from build123d import *

# Parameters (mm, degrees)
SKETCH1_W             = 50
SKETCH1_H             = 20
BOSS_EXTRUDE1_DEPTH   = 100
SKETCH2_R             = 3
BOSS_EXTRUDE2_DEPTH   = 5
M6_TAPPED_HOLE1_D     = 5
M6_TAPPED_HOLE1_DEPTH = 15
M6_TAPPED_HOLE1_TIP   = 1.502151548
SKETCH5_W             = 20
SKETCH5_H             = 30
BOSS_EXTRUDE3_DEPTH   = 120
M3_TAPPED_HOLE1_D     = 2.5
M3_TAPPED_HOLE1_DEPTH = 7.5
M3_TAPPED_HOLE1_TIP   = 0.751075774
SKETCH8_W             = 147.482871738
SKETCH8_H             = 30
CUT_EXTRUDE1_DEPTH    = 163.249807396
SKETCH9_R             = 3
BOSS_EXTRUDE4_DEPTH   = 5
M6_TAPPED_HOLE2_D     = 5
M6_TAPPED_HOLE2_DEPTH = 15
M6_TAPPED_HOLE2_TIP   = 1.502151548


with BuildPart() as part:
    # Sketch1 → Boss-Extrude1 (new body)
    with BuildSketch(Plane(origin=(0, 0, 0), x_dir=(1, 0, 0), z_dir=(0, 1, 0))):
        Rectangle(SKETCH1_W, SKETCH1_H)
    extrude(amount=BOSS_EXTRUDE1_DEPTH)

    # Sketch2 → Boss-Extrude2 (add)
    with BuildSketch(Plane.XZ):
        with Locations(Location((0, 5, 0), (0, 0, 270))):
            Circle(SKETCH2_R)
    extrude(amount=BOSS_EXTRUDE2_DEPTH)

    # M6 Tapped Hole1
    with Locations(Plane(origin=(0, 0, 0), x_dir=(-1, 0, 0), z_dir=(0, -1, 0))):
        with Locations((0, 5)):
            Hole(M6_TAPPED_HOLE1_D / 2, depth=M6_TAPPED_HOLE1_DEPTH)
            with Locations((0, 0, -(M6_TAPPED_HOLE1_DEPTH + M6_TAPPED_HOLE1_TIP / 2))):  # 118° drill point
                Cone(0, M6_TAPPED_HOLE1_D / 2, M6_TAPPED_HOLE1_TIP, mode=Mode.SUBTRACT)

    # Sketch5 → Boss-Extrude3 (add)
    with BuildSketch(Plane(origin=(25, 0, 0), x_dir=(0, 0, -1), z_dir=(1, 0, 0))):
        with Locations((0, 115)):
            Rectangle(SKETCH5_W, SKETCH5_H)
    extrude(amount=-BOSS_EXTRUDE3_DEPTH)

    # M3 Tapped Hole1
    with Locations(Plane.XY.offset(10)):
        with Locations((-63.4, 108), (-59.4, 112), (-67.4, 105)):
            Hole(M3_TAPPED_HOLE1_D / 2, depth=M3_TAPPED_HOLE1_DEPTH)
            with Locations((0, 0, -(M3_TAPPED_HOLE1_DEPTH + M3_TAPPED_HOLE1_TIP / 2))):  # 118° drill point
                Cone(0, M3_TAPPED_HOLE1_D / 2, M3_TAPPED_HOLE1_TIP, mode=Mode.SUBTRACT)

    # Sketch8 → Cut-Extrude1 (cut, through all)
    with BuildSketch(Plane.XY.offset(10)):
        with Locations((-48.741435869, 115)):
            Rectangle(SKETCH8_W, SKETCH8_H)
    extrude(amount=-CUT_EXTRUDE1_DEPTH, mode=Mode.SUBTRACT)

    # Sketch9 → Boss-Extrude4 (add)
    with BuildSketch(Plane(origin=(0, 100, 0), x_dir=(1, 0, 0), z_dir=(0, 1, 0))):
        with Locations((-10, 0)):
            Circle(SKETCH9_R)
    extrude(amount=BOSS_EXTRUDE4_DEPTH)

    # M6 Tapped Hole2
    with Locations(Plane(origin=(0, 100, 0), x_dir=(1, 0, 0), z_dir=(0, 1, 0))):
        with Locations((0, 0)):
            Hole(M6_TAPPED_HOLE2_D / 2, depth=M6_TAPPED_HOLE2_DEPTH)
            with Locations((0, 0, -(M6_TAPPED_HOLE2_DEPTH + M6_TAPPED_HOLE2_TIP / 2))):  # 118° drill point
                Cone(0, M6_TAPPED_HOLE2_D / 2, M6_TAPPED_HOLE2_TIP, mode=Mode.SUBTRACT)


solid = part.part
Geometry check sheet. Reference: the model listing, model coordinates, mm. A direction names the side the tool comes from. Give positions to 0.01 mm unless a question says otherwise; leave off trailing zeros. Write each loop counter-clockwise with the first axis right and the second up, starting at its lowest first coordinate (ties: lowest second). Pieces come first, ordered by that corner, then holes.
1) Release check for a two-part mould opening along X. For faces 3 (the face through (0.54, 92.4, 2.44)), 4 (the face through (-12.4, 102.5, 1.8)), 5 (the face through (0, 0, 0)) record: released by +X, released by -X, zero draft, split by the parting line, or undercut.
Values follow:
face 3: undercut
face 4: split by the parting line
face 5: zero draft
2) Go/stop test with flat-tipped pins: pin 1 Ø5 at (x, z) = (15, 0.5) entering from +Y; pin 2 Ø2 at (x, z) = (12, 7.5) entering from -Y. Record where each tip stops, or that it passes through.
Values follow:
pin 1: stops at y = 100
pin 2: stops at y = 0
3) Cross-section at B-B (x = -10). Record the boundary of the cut face in (y, z).
Values follow:
outline: (0, -10) - (100, -10) - (100, -3) - (105, -3) - (105, 3) - (100, 3) - (100, 10) - (0, 10) - close
4) Cross-section at C-C (x = 5). Record the boundary of the cut face in (y, z).
Values follow:
outline: (0, -10) - (100, -10) - (100, 10) - (0, 10) - close
5) Cross-section at A-A (z = 5). Record the boundary of the cut face in (x, y).
Values follow:
outline: (-25, 0) - (-3, 0) - (-3, -5) - (3, -5) - (3, 0) - (25, 0) - (25, 100) - (-25, 100) - close
6) Set-up check for faces 1 (the face through (0.9, -2.46, 2.14)), 2 (the face through (0, -5, 5)): record each of +Z, -Z, +X, -X, +Y, -Y from which the full face is reachable in a straight line by a thin tool's end or side.
Values follow:
face 1: -Y
face 2: +Z, -Z, +X, -X, -Y
7) Thickness scan on line 1 (Z direction, x = 0, y = 92.25); line 2 (Y direction, x = -12.5, z = 4.5); line 3 (X direction, y = 93.5, z = 1.75). Record the ranges inside material, lowest first.
Values follow:
line 1: z = -10 to -2.5, 2.5 to 10
line 2: y = 0 to 100
line 3: x = -25 to -1.79, 1.79 to 25
